Check sheet for the modelled part. Datum: model origin and axes. Units: mm. Face numbers are marked on the shaded views. A direction names the side the tool comes from. Coordinates: 2 decimals unless noted, no trailing zeros. Write each loop counter-clockwise with the first axis right and the second up, starting at its lowest first coordinate (ties: lowest second). Pieces come first, ordered by that corner, then holes. Notation, with made-up numbers: (29.25, 39) -> (66.25, 39) arc R21 ccw to (66.25, 47) -> close; hole circle Ø8 at (-32.5, -3). An arc over 180 degrees is marked (long way). One line per item, written item: value. Start each with the question number.
1) Sectioned sample at D-D on z = -7. Enter the section's corners in (x, y), plus the area to 3 significant figures.
2) Draft check along Z on the marked faces 1, 2 and 3. Enter one of: +Z half, -Z half, draft (parallel to the pull), parting line (faces both ways), or undercut.
3) Set-up check for the marked faces 4, 5, 6 and 7: record each of +Z, -Z, +X, -X, +Y, -Y from which the full face is reachable in a straight line by a thin tool's end or side.
4) Sectioned sample at B-B on y = 0. Enter the section's corners in (x, z), plus the area to 3 significant figures.
5) Sectioned sample at C-C on x = 36. Enter the section's corners in (y, z), plus the area to 3 significant figures.
6) Sectioned sample at A-A on z = 0. Enter the section's corners in (x, y).
7) Scan lines: line 1 along Z through (x, y) = (12, 0); line 2 along Z through (x, y) = (31, 0); line 3 along X through (y, z) = (-7.75, -0.5). Record each from-to range of solid material in increasing order. Write a range as [from, to].
8) Gauge pin test, flat ends, axial feed: P1, Ø8, axis at x = 21.5, y = -1.5, coming from the +Z side; P2, Ø3, axis at x = 30.5, y = 5.5, coming from the +Z side; P3, Ø6, axis at x = 24, z = 0, coming from the +Y side; P4, Ø1.5, axis at x = 24.5, y = -5.5, coming from the -Z side. Record the tip position at first contact, or that the pin passes through.
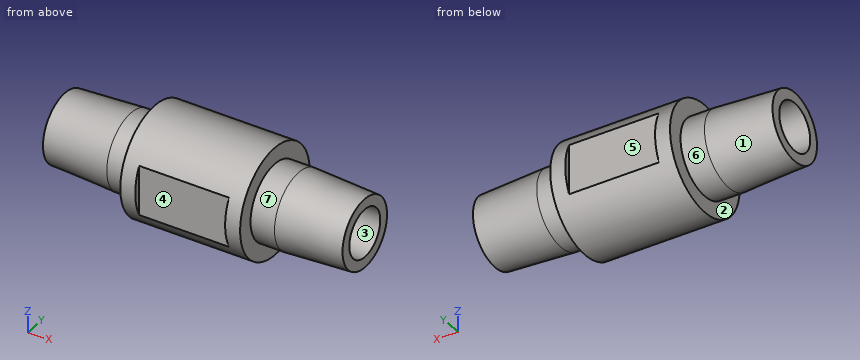
```python
from build123d import *

# Parameters (mm, degrees)
SKETCH_2_OUTSIDE_W   = 31.222
SKETCH_2_OUTSIDE_H   = 31.222
SKETCH_2_OUTSIDE_W_2 = 20.905852418
SKETCH_2_OUTSIDE_H_2 = 16
CUT_EXTRUDE_1_DEPTH  = 7.5


with BuildPart() as part:
    # 草图1 → 旋转1 (revolve)
    with BuildSketch(Plane.XY, mode=Mode.PRIVATE) as revolve_1_sk:
        Polygon((0, 4), (0, 5.75), (11, 6.3), (15, 6.3), (15, 9), (35, 9), (35, 6.3), (39, 6.3), (50, 5.75), (50, 4), align=None)
    revolve(revolve_1_sk.sketch.rotate(Axis((0, 0, 0), (1, 0, 0)), 180), axis=Axis((0, 0, 0), (1, 0, 0)))

    # 草图2 outside → 切除-拉伸1 (cut, symmetric)
    with BuildSketch(Plane.ZY.offset(-25)):
        Rectangle(SKETCH_2_OUTSIDE_W, SKETCH_2_OUTSIDE_H)
        Rectangle(SKETCH_2_OUTSIDE_W_2, SKETCH_2_OUTSIDE_H_2, mode=Mode.SUBTRACT)
    extrude(amount=CUT_EXTRUDE_1_DEPTH, both=True, mode=Mode.SUBTRACT)


solid = part.part
```
Answers:
1. outline: (15, -5.66) -> (35, -5.66) -> (35, 5.66) -> (15, 5.66) -> close
1. area: 226 mm2
2. face 1: parting line
2. face 2: draft
2. face 3: undercut
3. face 4: +Z, -Z, -Y
3. face 5: +Z, -Z, +Y
3. face 6: -X
3. face 7: +X
4. outline: (0, -5.75) -> (11, -6.3) -> (15, -6.3) -> (15, -9) -> (35, -9) -> (35, -6.3) -> (39, -6.3) -> (50, -5.75) -> (50, -4) -> (0, -4) -> close; (0, 4) -> (50, 4) -> (50, 5.75) -> (39, 6.3) -> (35, 6.3) -> (35, 9) -> (15, 9) -> (15, 6.3) -> (11, 6.3) -> (0, 5.75) -> close
4. area: 326 mm2
5. outline: circle Ø12.6 at (0, 0); hole circle Ø8 at (0, 0)
5. area: 74.4 mm2
6. outline: (0, -5.75) -> (11, -6.3) -> (15, -6.3) -> (15, -9) -> (17.5, -9) -> (17.5, -8) -> (32.5, -8) -> (32.5, -9) -> (35, -9) -> (35, -6.3) -> (39, -6.3) -> (50, -5.75) -> (50, -4) -> (0, -4) -> close; (0, 4) -> (50, 4) -> (50, 5.75) -> (39, 6.3) -> (35, 6.3) -> (35, 9) -> (32.5, 9) -> (32.5, 8) -> (17.5, 8) -> (17.5, 9) -> (15, 9) -> (15, 6.3) -> (11, 6.3) -> (0, 5.75) -> close
7. line 1: z = [-6.3, -4], [4, 6.3]
7. line 2: z = [-9, -4], [4, 9]
7. line 3: x = [15, 35]
8. P1: stops at z = 9
8. P2: stops at z = 8.06
8. P3: stops at y = 8
8. P4: stops at z = -7.64
